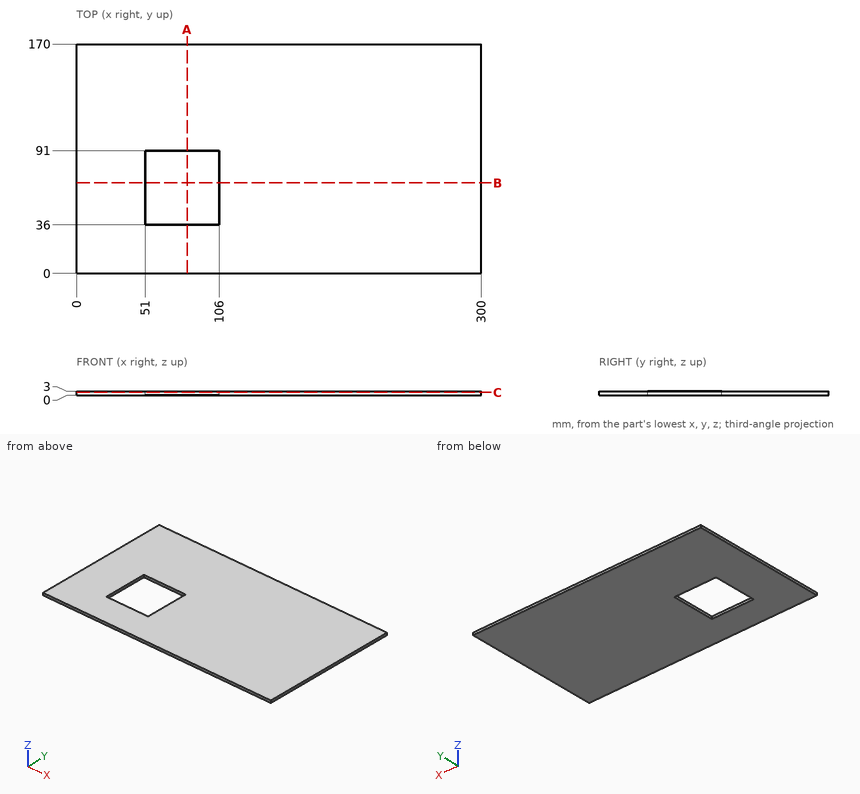
Design review of the part shown in the three views and the two pictorial views. Dimensions are in mm from the part's minimum x, y and z. Round coordinates to 2 decimals unless told otherwise and drop trailing zeros. Write each loop counter-clockwise with the first axis right and the second up, starting at its lowest first coordinate (ties: lowest second). Pieces come first, ordered by that corner, then holes. Notation, with made-up numbers: M 3.25,66 L 29.25,66 A18 ccw 29.25,75 Z; hole C -5,-32.5 d4. An arc over 180 degrees is marked long. Use a Markdown table: item, result. Add a question column.
Q1. We need section C-C, the plane z = 2.3. State the section outline as (x, y) points, plus the area to 3 significant figures.
Q2. We need section A-A, the plane x = 82. State the section outline as (y, z) points.
Q3. To check wall thickness, follow line 1 (Y direction, x = 99, z = 1.3); line 2 (X direction, y = 75.5, z = 2.75). State the ranges of each line that lie inside material, in increasing order.
Q4. Insertion check: pin 1 (12 mm diameter, centred on x = 186, y = 52, fed in from -Z). The pin has a flat end and moves straight along its axis. Give the tip position at first contact, or say it passes through.
Q5. We need section B-B, the plane y = 67. State the section outline as (x, z) points, plus the area to 3 significant figures.
Findings below:
| question | item | result |
|---|---|---|
| 1 | outline | M 0,0 L 300,0 L 300,170 L 0,170 Z; hole M 51,36 L 106,36 L 106,91 L 51,91 Z |
| 1 | area | 48,000 mm² |
| 2 | outline | M 0,0 L 36,0 L 36,3 L 0,3 Z; M 91,0 L 170,0 L 170,3 L 91,3 Z |
| 3 | line 1 | y = 0 to 36, 91 to 170 |
| 3 | line 2 | x = 0 to 51, 106 to 300 |
| 4 | pin 1 | stops at z = 0 |
| 5 | outline | M 0,0 L 51,0 L 51,3 L 0,3 Z; M 106,0 L 300,0 L 300,3 L 106,3 Z |
| 5 | area | 735 mm² |
